Could you check a few things on this model? Use its own coordinates, in mm. A direction names the side the tool comes from. Round coordinates to 2 decimals unless told otherwise and drop trailing zeros. Loops run counter-clockwise (first coordinate to the right, second up) from the corner with the lowest first, then second, coordinate; pieces in that order, holes last.
from build123d import *

# Parameters (mm, degrees)
EXTRUDE_1_DEPTH     = 30
SHELL_1_T           = -1.5
EXTRUDE_2_DEPTH     = 1.5
CUT_EXTRUDE_1_DEPTH = 1.5
FILLET_1_R          = 3
SKETCH_4_W          = 110
SKETCH_4_H          = 4.5
CUT_EXTRUDE_2_DEPTH = 30


with BuildPart() as part:
    # 草图1 → 凸台-拉伸1 (new body)
    with BuildSketch(Plane.XY):
        with BuildLine():
            Line((0.440140845, 24.99612522), (142.396126761, 22.496512698))
            ThreePointArc((142.396126761, 22.496512698), (164.5, 0), (142.396126761, -22.496512698))
            Line((142.396126761, -22.496512698), (0.440140845, -24.99612522))
            ThreePointArc((0.440140845, -24.99612522), (-25, 0), (0.440140845, 24.99612522))
        make_face()
    extrude(amount=EXTRUDE_1_DEPTH)

    # 抽壳1
    shell_1_openings = [part.faces().sort_by_distance(p)[0] for p in [
        (68.129004911, 0, 0),
    ]]
    offset(amount=SHELL_1_T, openings=shell_1_openings, kind=Kind.INTERSECTION)

    # 草图2 → 凸台-拉伸2 (add)
    with BuildSketch(Plane(origin=(0, 0, 0), x_dir=(-1, 0, 0), z_dir=(0, 0, -1))):
        Polygon((-30, 24.475624492), (-30, 35), (-15, 35), (-15, 24.739749936), align=None)
    extrude_2 = extrude(amount=-EXTRUDE_2_DEPTH)

    # 草图3 → 切除-拉伸1 (cut)
    with BuildSketch(Plane.XY.offset(1.5)):
        with BuildLine():
            Line((26.5, 27.9), (18.5, 27.9))
            ThreePointArc((18.5, 27.9), (16.4, 30), (18.5, 32.1))
            Line((18.5, 32.1), (26.5, 32.1))
            ThreePointArc((26.5, 32.1), (28.6, 30), (26.5, 27.9))
        make_face()
    cut_extrude_1 = extrude(amount=-CUT_EXTRUDE_1_DEPTH, mode=Mode.SUBTRACT)

    # 镜向1: 凸台-拉伸2, 切除-拉伸1 across plane
    add(extrude_2.mirror(Plane.ZX))
    add(cut_extrude_1.mirror(Plane.ZX), mode=Mode.SUBTRACT)

    # 圆角1
    fillet_1_edges = [part.edges().sort_by_distance(p)[0] for p in [
        (164.5, 0, 30),
        (71.418133803, 23.746318959, 30),
        (-23.5, 0, 28.5),
        (71.391725352, -22.246551446, 28.5),
        (163, 0, 28.5),
        (71.391725352, 22.246551446, 28.5),
        (30, 35, 0.75),
        (15, 35, 0.75),
        (-25, 0, 30),
        (15, -35, 0.75),
        (30, -35, 0.75),
        (71.418133803, -23.746318959, 30),
    ]]
    fillet(fillet_1_edges, radius=FILLET_1_R)

    # 草图4 → 切除-拉伸2 (cut, symmetric)
    with BuildSketch(Plane(origin=(0, 0, 0), x_dir=(1, 0, 0), z_dir=(0, 1, 0))):
        with Locations((109.5, -2.25)):
            Rectangle(SKETCH_4_W, SKETCH_4_H)
    extrude(amount=CUT_EXTRUDE_2_DEPTH, both=True, mode=Mode.SUBTRACT)


solid = part.part
Item 1: If we section it at A-A, the plane y = -30: Please give me the cut outline in (x, z), then the cut area to 3 significant figures.
Results list:
outline: (15, 0) - (16.4, 0) - (16.4, 1.5) - (15, 1.5) - close; (28.6, 0) - (30, 0) - (30, 1.5) - (28.6, 1.5) - close
area: 4.20 mm2
Item 2: We'd pull the mould along X, two halves only. Please class faces 1 (the cylindrical face through (72.37, 21.37, 27.6)), 2 (the cylindrical face through (164.495, 0.489, 15.592)), 3 (the flat face through (71, 0, 30)): released by +X, released by -X, zero draft, split by the parting line, or undercut.
Results list:
face 1: undercut
face 2: released by +X
face 3: zero draft
Item 3: If I drill on line 1 along Y through (x, z) = (55, 21); line 2 along Y through (x, z) = (53.5, 2); line 3 along Z through (x, y) = (59.5, 14), over which ranges is the centre line in solid material (lowest first)?
Results list:
line 1: y = -24.04 to -22.54, 22.54 to 24.04
line 2: y = -24.06 to -22.56, 22.56 to 24.06
line 3: z = 28.5 to 30
Item 4: If we section it at B-B, the plane z = 6.25: Please give me the cut outline in (x, y).
Results list:
outline: (0.44, -25) - (142.4, -22.5) arc R22.5 ccw to (142.4, 22.5) - (0.44, 25) arc R25 ccw (long way) to start; hole (0.41, -23.5) - (142.37, -21) arc R21 ccw to (142.37, 21) - (0.41, 23.5) arc R23.5 ccw (long way) to start
Item 5: For faces 4 (the flat face through (105, -23, 4.5)), 5 (the cylindrical face through (163, 0, 15)), 6 (the cylindrical face through (70.409, -22.908, 29.098)), which set-ups out of +Z, -Z, +X, -X, +Y, -Y let a thin tool reach every point of the face, with its end or its side?
Results list:
face 4: -Z, +X, +Y, -Y
face 5: -Z
face 6: +Z, +X, -Y
Item 6: Will these pins go through, and if not, where does the flat tip stop? pin 1 (11.5 mm diameter, centred on x = 20, y = -29.5, fed in from +Z); pin 2 (14.5 mm diameter, centred on x = 85.5, y = 2, fed in from -Z); pin 3 (1.2 mm diameter, centred on y = -27, z = 0.5, fed in from +X).
Results list:
pin 1: stops at z = 29.14
pin 2: stops at z = 28.5
pin 3: stops at x = 30
